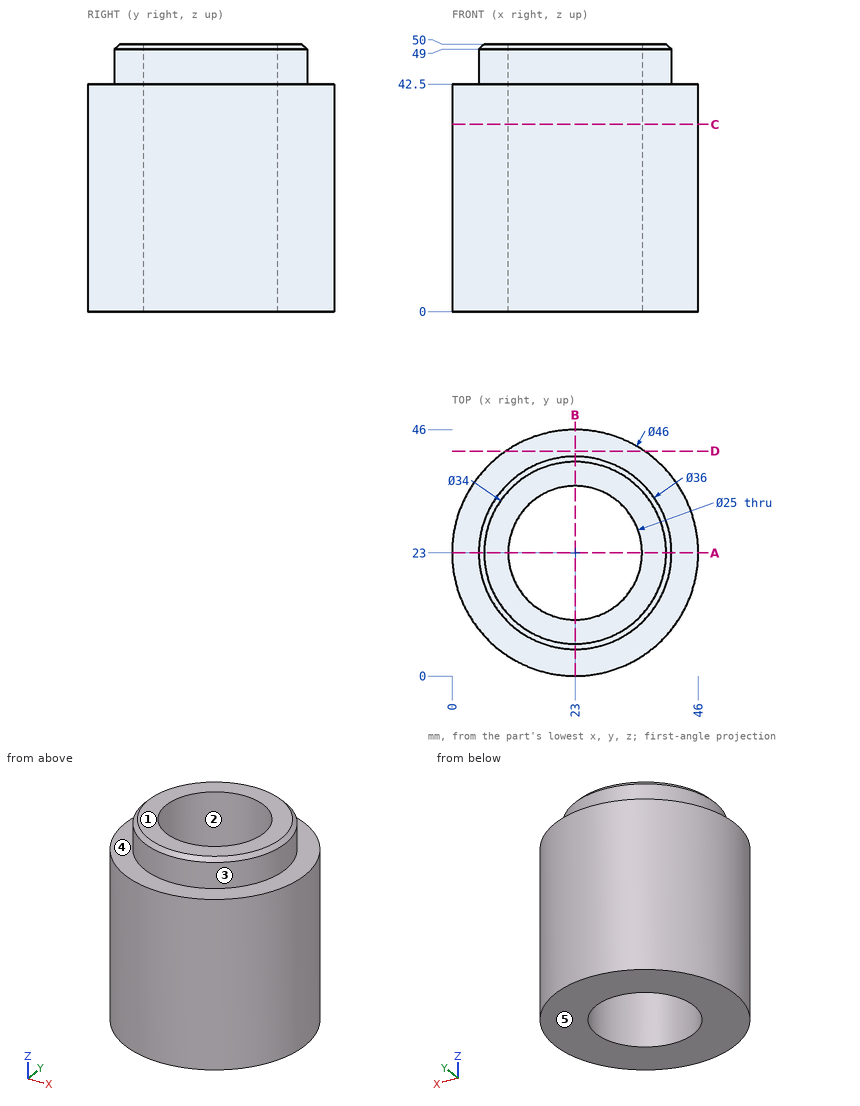
The figure shows three views and two pictorial views of one solid part (mm, origin at its lowest corner). Answer the questions. A direction names the side the tool comes from. Coordinates: 2 decimals unless noted, no trailing zeros. Loops run counter-clockwise (first coordinate to the right, second up) from the corner with the lowest first, then second, coordinate; pieces in that order, holes last. Notation, with made-up numbers: (17.5, 67) - (35.5, 67) arc R21 cw to (35.5, 72) - close; hole circle Ø11 at (-20.75, 4). An arc over 180 degrees is marked (long way). Use a Markdown table: item, result. Add a question column.
1) The mould has two halves that part along X. Classify the marked faces 1, 2 and 3: released by +X, released by -X, zero draft, split by the parting line, or undercut.
2) The part is cut by section C-C, the plane z = 35. Give the vertices of the cut face in (x, y), and give its area (3 significant figures).
3) For the marked faces 4 and 5, determine the directions among +Z, -Z, +X, -X, +Y, -Y from which every point of the face is accessible in a straight line to the end or side of a thin tool.
4) The part is cut by section A-A, the plane y = 23. Give the vertices of the cut face in (x, z).
5) Find the intervals of material crossed by line 1 (Y direction, x = 23, z = 29); line 2 (Z direction, x = 32.5, y = 43.5); line 3 (X direction, y = 13.5, z = 22.5), in increasing order.
6) The part is cut by section D-D, the plane y = 42. Give the vertices of the cut face in (x, z), and give its area (3 significant figures).
7) Given pin 1 (12 mm diameter, centred on x = 5, z = 24.5, fed in from +Y); pin 2 (1 mm diameter, centred on y = 39.5, z = 24, fed in from -X); pin 3 (1.5 mm diameter, centred on x = 27.5, z = 5.5, fed in from +Y), each flat-ended and moving along its own axis, determine where each tip first touches the part or whether it passes through.
Here are the results:
| question | item | result |
|---|---|---|
| 1 | face 1 | zero draft |
| 1 | face 2 | undercut |
| 1 | face 3 | split by the parting line |
| 2 | outline | circle Ø46 at (23, 23); hole circle Ø25 at (23, 23) |
| 2 | area | 1,170 mm^2 |
| 3 | face 4 | +Z |
| 3 | face 5 | -Z, +X, -X, +Y, -Y |
| 4 | outline | (0, 0) - (10.5, 0) - (10.5, 50) - (6, 50) - (5, 49) - (5, 42.5) - (0, 42.5) - close; (35.5, 0) - (46, 0) - (46, 42.5) - (41, 42.5) - (41, 49) - (40, 50) - (35.5, 50) - close |
| 5 | line 1 | y = 0 to 10.5, 35.5 to 46 |
| 5 | line 2 | z = 0 to 42.5 |
| 5 | line 3 | x = 2.05 to 14.88, 31.12 to 43.95 |
| 6 | outline | (10.04, 0) - (35.96, 0) - (35.96, 42.5) - (10.04, 42.5) - close |
| 6 | area | 1,100 mm^2 |
| 7 | pin 1 | stops at y = 42.62 |
| 7 | pin 2 | stops at x = 6.48 |
| 7 | pin 3 | stops at y = 45.69 |
